Geometry: final body of the model. Coordinates: model frame, mm. Face numbers are marked on the shaded views. A direction names the side the tool comes from. Round coordinates to 2 decimals unless told otherwise and drop trailing zeros. Order: outer loops, then holes, each group sorted by start corner. A loop starts at its lowest first (then second) coordinate and runs counter-clockwise, first axis right, second up. Notation, with made-up numbers: (67, -29) -> (77, -29) arc R20 cw to (77, 2) -> close; hole circle Ø9 at (62, 24.5). An arc over 180 degrees is marked (long way). Put each result on its own line as item: value.
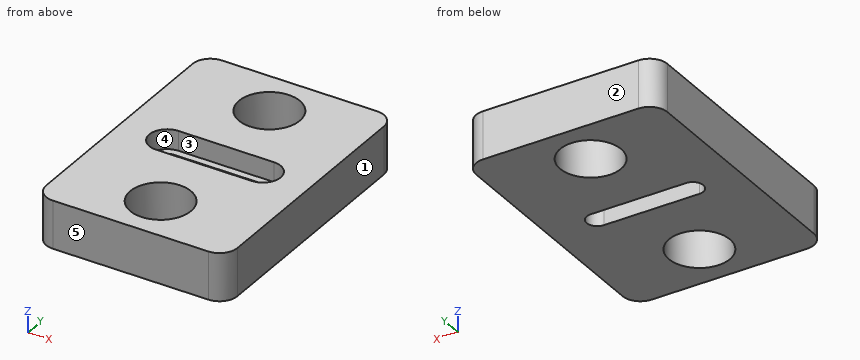
```python
from build123d import *

# Parameters (mm, degrees)
SKETCH1_W           = 32
SKETCH1_H           = 45
BOSS_EXTRUDE1_DEPTH = 8
CUT_EXTRUDE1_DEPTH  = 29.744564704
CUT_EXTRUDE2_DEPTH  = 3.3
FILLET1_R           = 3
M12_TAPPED_HOLE2_D  = 10.2


with BuildPart() as part:
    # Sketch1 → Boss-Extrude1 (new body)
    with BuildSketch(Plane.XY):
        Rectangle(SKETCH1_W, SKETCH1_H)
    extrude(amount=BOSS_EXTRUDE1_DEPTH)

    # Sketch5 → Cut-Extrude1 (cut, through all)
    with BuildSketch(Plane.XY.offset(8)):
        with BuildLine():
            Line((-8, 1.75), (8, 1.75))
            ThreePointArc((8, 1.75), (9.75, 0), (8, -1.75))
            Line((8, -1.75), (-8, -1.75))
            ThreePointArc((-8, -1.75), (-9.75, 0), (-8, 1.75))
        make_face()
    extrude(amount=-CUT_EXTRUDE1_DEPTH, mode=Mode.SUBTRACT)

    # Sketch6 → Cut-Extrude2 (cut)
    with BuildSketch(Plane.XY.offset(8)):
        with BuildLine():
            Line((-8, 3), (8, 3))
            ThreePointArc((8, 3), (11, 0), (8, -3))
            Line((8, -3), (-8, -3))
            ThreePointArc((-8, -3), (-11, 0), (-8, 3))
        make_face()
    extrude(amount=-CUT_EXTRUDE2_DEPTH, mode=Mode.SUBTRACT)

    # Fillet1
    fillet1_edges = [part.edges().sort_by_distance(p)[0] for p in [
        (-16, 22.5, 4),
        (16, 22.5, 4),
        (16, -22.5, 4),
        (-16, -22.5, 4),
    ]]
    fillet(fillet1_edges, radius=FILLET1_R)

    # M12 Tapped Hole2 (through all)
    with Locations(Plane.XY.offset(8)):
        with Locations((0, -14.5), (0, 14.5)):
            Hole(M12_TAPPED_HOLE2_D / 2)


solid = part.part
```
1. Cut plane B-B on y = 0. Return loops of the section in (x, z).
Ans:
outline: (-16, 0) -> (-9.75, 0) -> (-9.75, 4.7) -> (-11, 4.7) -> (-11, 8) -> (-16, 8) -> close; (9.75, 0) -> (16, 0) -> (16, 8) -> (11, 8) -> (11, 4.7) -> (9.75, 4.7) -> close
2. Cut plane C-C on z = 5.5. Return loops of the section in (x, y), and give its area (3 significant figures).
Ans:
outline: (-16, -19.5) arc R3 ccw to (-13, -22.5) -> (13, -22.5) arc R3 ccw to (16, -19.5) -> (16, 19.5) arc R3 ccw to (13, 22.5) -> (-13, 22.5) arc R3 ccw to (-16, 19.5) -> close; hole (-8, -3) -> (8, -3) arc R3 ccw to (8, 3) -> (-8, 3) arc R3 ccw to start; hole circle Ø10.2 at (0, -14.5); hole circle Ø10.2 at (0, 14.5)
area: 1,140 mm²
3. Cut plane D-D on x = 0. Return loops of the section in (y, z), and give its area (3 significant figures).
Ans:
outline: (-22.5, 0) -> (-19.6, 0) -> (-19.6, 8) -> (-22.5, 8) -> close; (-9.4, 0) -> (-1.75, 0) -> (-1.75, 4.7) -> (-3, 4.7) -> (-3, 8) -> (-9.4, 8) -> close; (1.75, 0) -> (9.4, 0) -> (9.4, 8) -> (3, 8) -> (3, 4.7) -> (1.75, 4.7) -> close; (19.6, 0) -> (22.5, 0) -> (22.5, 8) -> (19.6, 8) -> close
area: 161 mm²
4. Set-up query: the marked faces 4 and 5. Return all of +Z, -Z, +X, -X, +Y, -Y with unobstructed straight access to the full face (end or side cutting, diameter ignored); none if empty.
Ans:
face 4: +Z
face 5: +Z, -Z, +X, -X, -Y
5. Cut plane A-A on x = -6.5. Return loops of the section in (y, z), and give its area (3 significant figures).
Ans:
outline: (-22.5, 0) -> (-1.75, 0) -> (-1.75, 4.7) -> (-3, 4.7) -> (-3, 8) -> (-22.5, 8) -> close; (1.75, 0) -> (22.5, 0) -> (22.5, 8) -> (3, 8) -> (3, 4.7) -> (1.75, 4.7) -> close
area: 324 mm²
6. Material intervals for probe 1 along Y at (x, z) = (0, 4.5); probe 2 along Y at (x, z) = (0, 5); probe 3 along X at (y, z) = (0, 5.25), sorted ascending.
Ans:
probe 1: -22.5 to -19.6, -9.4 to -1.75, 1.75 to 9.4, 19.6 to 22.5
probe 2: -22.5 to -19.6, -9.4 to -3, 3 to 9.4, 19.6 to 22.5
probe 3: -16 to -11, 11 to 16
7. Draft query along X for the marked faces 1, 2 and 3. Return one class per face: +X half, -X half, draft (parallel to the pull), parting line (faces both ways), or undercut.
Ans:
face 1: +X half
face 2: draft
face 3: undercut
